The drawing under review shows one solid part. Ordinate dimensions are in mm from its lowest x, y, z. A direction names the side the tool comes from. Coordinates: 2 decimals unless noted, no trailing zeros. Loops run counter-clockwise (first coordinate to the right, second up) from the corner with the lowest first, then second, coordinate; pieces in that order, holes last. Notation, with made-up numbers: M 59,-4.75 L 111,-4.75 A17 ccw 111,28.25 Z; hole C -31.75,-28 d3. An arc over 180 degrees is marked long. Return JSON: item names as keys, results as strings.
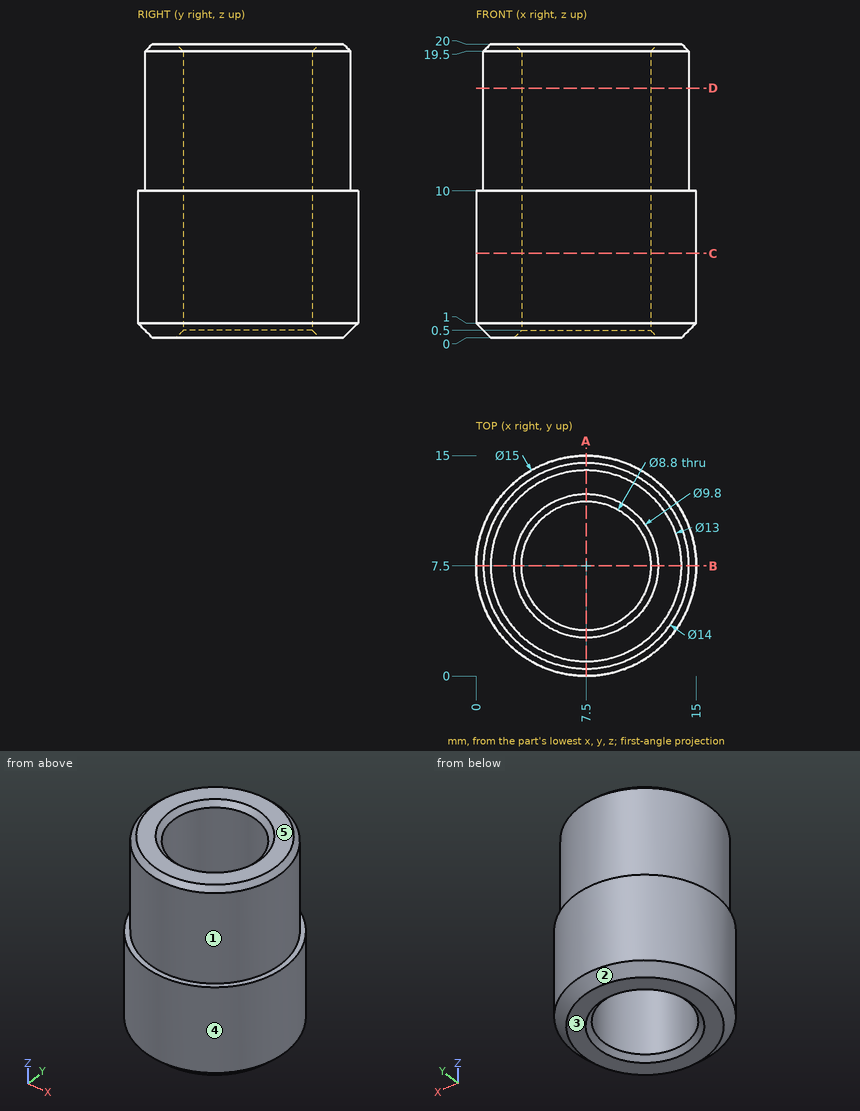
1. Machinability: for the marked faces 1 and 2, which of the approach directions +Z, -Z, +X, -X, +Y, -Y give a long, thin tool a straight path to every point of the face, cutting with its end or side? Answer none if there is none.
Check values:
{"face 1": "+Z", "face 2": "-Z"}
2. Add section C-C on z = 5.75. Give the boundary of the cut face in (x, y).
Check values:
{"outline": "C 7.5,7.5 d15; hole C 7.5,7.5 d8.8"}
3. Add section D-D on z = 17. Give the boundary of the cut face in (x, y), plus the area to 3 significant figures.
Check values:
{"outline": "C 7.5,7.5 d14; hole C 7.5,7.5 d8.8", "area": "93.1 mm²"}
4. The part is to be moulded in two halves that separate along Z. For the marked faces 3, 4 and 5, say which applies: released by +Z, released by -Z, zero draft, split by the parting line, or undercut.
Check values:
{"face 3": "released by -Z", "face 4": "zero draft", "face 5": "released by +Z"}
5. Add section A-A on x = 7.5. Give the boundary of the cut face in (y, z).
Check values:
{"outline": "M 0,1 L 1,0 L 2.6,0 L 3.1,0.5 L 3.1,19.5 L 2.6,20 L 1,20 L 0.5,19.5 L 0.5,10 L 0,10 Z; M 11.9,0.5 L 12.4,0 L 14,0 L 15,1 L 15,10 L 14.5,10 L 14.5,19.5 L 14,20 L 12.4,20 L 11.9,19.5 Z"}
6. Insertion check: pin 1 Ø1.5 at (x, z) = (12.5, 8) entering from -Y; pin 2 Ø5 at (x, y) = (1.5, 7.5) entering from -Z; pin 3 Ø5 at (x, z) = (5.5, 17.5) entering from +Y; pin 4 Ø2 at (x, z) = (8, 16.5) entering from -Y. Each pin has a flat end and moves straight along its axis. Give the tip position at first contact, or say it passes through.
Check values:
{"pin 1": "y = 1.32", "pin 2": "z = 0", "pin 3": "y = 14.5", "pin 4": "y = 0.5"}
7. To check wall thickness, follow line 1 (Y direction, x = 7.5, z = 14); line 2 (Y direction, x = 7.5, z = 9.5); line 3 (X direction, y = 4.5, z = 8). State the ranges of each line that lie inside material, in increasing order.
Check values:
{"line 1": "0.5 to 3.1, 11.9 to 14.5", "line 2": "0 to 3.1, 11.9 to 15", "line 3": "0.63 to 4.28, 10.72 to 14.37"}
